```python
from build123d import *

# Parameters (mm, degrees)
SKETCH_1_W          = 46
SKETCH_1_H          = 30
EXTRUDE_1_DEPTH     = 10
SKETCH_2_W          = 41
SKETCH_2_H          = 30
CUT_EXTRUDE_1_DEPTH = 1.5


with BuildPart() as part:
    # 草图1 → 凸台-拉伸1 (new body)
    with BuildSketch(Plane.XY):
        Rectangle(SKETCH_1_W, SKETCH_1_H)
    extrude(amount=EXTRUDE_1_DEPTH)

    # 草图2 → 切除-拉伸1 (cut)
    with BuildSketch(Plane.XY.offset(10)):
        Rectangle(SKETCH_2_W, SKETCH_2_H)
    extrude(amount=-CUT_EXTRUDE_1_DEPTH, mode=Mode.SUBTRACT)

    # 草图3 → M4 螺纹孔1 (revolve, cut)
    with BuildSketch(Plane(origin=(16, 15, 4.5), x_dir=(0, 0, 1), z_dir=(1, 0, 0))):
        Polygon((0, 0), (0, 9.091420021), (1.65, 8.1), (1.65, 0.375), (2.025, 0), align=None)
    hole_wizard_m4_1 = revolve(axis=Axis((16, 21.35, 4.5), (0, -1, 0)), mode=Mode.SUBTRACT)

    # 镜向1: M4 螺纹孔1 across plane
    add(hole_wizard_m4_1.mirror(Plane(origin=(0, 0, 0), x_dir=(0, 0, 1), z_dir=(1, 0, 0))), mode=Mode.SUBTRACT)


solid = part.part
```
The listing builds one solid part. Answer for the finished solid, in the listing's coordinates (mm). A direction names the side the tool comes from. Round coordinates to 2 decimals unless told otherwise and drop trailing zeros. Order: outer loops, then holes, each group sorted by start corner. A loop starts at its lowest first (then second) coordinate and runs counter-clockwise, first axis right, second up. Notation, with made-up numbers: (-32, -31) - (10, -31) arc R10 ccw to (10, -22) - close; hole circle Ø6 at (35, 1). An arc over 180 degrees is marked (long way). Put each result on its own line as item: value. Start each with the question number.
(1) Given P1, Ø1, axis at x = -16, y = 0.5, coming from the +Z side, flat-ended and moving along its own axis, determine where the tip first touches the part or whether it passes through.
(2) Straight lines are drawn through the part: probe 1 along X at (y, z) = (10, 4.5); probe 2 along X at (y, z) = (12.25, 5.75); probe 3 along X at (y, z) = (-5, 8.75). For each, find the intervals that lie inside material, in ascending order. Write a range as from..to.
(3) For faces 1 (the flat face through (-22, 0, 10)), 2 (the flat face through (-20.5, 0, 9)), 3 (the cylindrical face through (-15.93, 10.82, 2.85)), determine the directions among +Z, -Z, +X, -X, +Y, -Y from which every point of the face is accessible in a straight line to the end or side of a thin tool.
(4) Determine the mould class of faces 4 (the flat face through (20.5, 0, 9)), 5 (the cylindrical face through (15.93, 10.82, 2.85)), 6 (the flat face through (0, 0, 0)) for opening direction Z: released by +Z, released by -Z, zero draft, split by the parting line, or undercut.
(5) Find section B-B (x = -9). Give the vertices of the cut face in (y, z).
(6) Find section A-A (y = -1.5). Give the vertices of the cut face in (x, z).
Reply:
1. P1: z = 8.5
2. probe 1: -23..-17.65, -14.35..14.35, 17.65..23
2. probe 2: -23..-17.08, -14.92..14.92, 17.08..23
2. probe 3: -23..-20.5, 20.5..23
3. face 1: +Z, +X, -X, +Y, -Y
3. face 2: +Z, +Y, -Y
3. face 3: +Y
4. face 4: zero draft
4. face 5: undercut
4. face 6: released by -Z
5. outline: (-15, 0) - (15, 0) - (15, 8.5) - (-15, 8.5) - close
6. outline: (-23, 0) - (23, 0) - (23, 10) - (20.5, 10) - (20.5, 8.5) - (-20.5, 8.5) - (-20.5, 10) - (-23, 10) - close
